```python
from build123d import *

# Parameters (mm, degrees)
BOSS_EXTRUDE1_DEPTH = 50
FILLET1_R           = 3
SKETCH3_R           = 2.5
CUT_EXTRUDE1_DEPTH  = 3
SKETCH4_R           = 1.5
CUT_EXTRUDE2_DEPTH  = 52.816130281
SKETCH5_R           = 1.5
CUT_EXTRUDE3_DEPTH  = 52.816130281
FILLET5_R           = 3
FILLET6_R           = 3
FILLET7_R           = 1


with BuildPart() as part:
    # Sketch1 → Boss-Extrude1 (new body)
    with BuildSketch(Plane.XY):
        Polygon((-4.736842105, 0), (-4.736842105, 6), (13.263157895, 6), (13.263157895, 0.55), (7.263157895, 0.55), (7.263157895, 0), align=None)
    extrude(amount=BOSS_EXTRUDE1_DEPTH)

    # Fillet1
    fillet1_edges = [part.edges().sort_by_distance(p)[0] for p in [
        (7.263157895, 0.275, 50),
    ]]
    fillet(fillet1_edges, radius=FILLET1_R)

    # Sketch3 → Cut-Extrude1 (cut)
    with BuildSketch(Plane(origin=(0, 6, 0), x_dir=(1, 0, 0), z_dir=(0, 1, 0))):
        with Locations(Location((0.263157895, -10, 0), (0, 0, 180))):
            Circle(SKETCH3_R)
        with Locations(Location((0.263157895, -40, 0), (0, 0, 180))):
            Circle(SKETCH3_R)
    extrude(amount=-CUT_EXTRUDE1_DEPTH, mode=Mode.SUBTRACT)

    # Sketch4 → Cut-Extrude2 (cut, through all)
    with BuildSketch(Plane(origin=(0, 3, 0), x_dir=(1, 0, 0), z_dir=(0, 1, 0))):
        with Locations(Location((0.263157895, -40, 0), (0, 0, 180))):
            Circle(SKETCH4_R)
    extrude(amount=-CUT_EXTRUDE2_DEPTH, mode=Mode.SUBTRACT)

    # Sketch5 → Cut-Extrude3 (cut, through all)
    with BuildSketch(Plane(origin=(0, 3, 0), x_dir=(1, 0, 0), z_dir=(0, 1, 0))):
        with Locations(Location((0.263157895, -10, 0), (0, 0, 180))):
            Circle(SKETCH5_R)
    extrude(amount=-CUT_EXTRUDE3_DEPTH, mode=Mode.SUBTRACT)

    # Fillet5
    fillet5_edges = [part.edges().sort_by_distance(p)[0] for p in [
        (7.263157895, 0.275, 0),
    ]]
    fillet(fillet5_edges, radius=FILLET5_R)

    # Fillet6
    fillet6_edges = [part.edges().sort_by_distance(p)[0] for p in [
        (-4.736842105, 3, 50),
        (-4.736842105, 3, 0),
    ]]
    fillet(fillet6_edges, radius=FILLET6_R)

    # Fillet7
    fillet7_edges = [part.edges().sort_by_distance(p)[0] for p in [
        (13.263157895, 6, 25),
        (5.763157895, 6, 50),
        (-4.736842105, 6, 25),
        (-3.858162449, 6, 49.121320344),
        (-3.858162449, 6, 0.878679656),
        (5.763157895, 6, 0),
    ]]
    fillet(fillet7_edges, radius=FILLET7_R)


solid = part.part
```
Part model, mm, in its own coordinate system. A direction names the side the tool comes from. Round coordinates to 2 decimals unless told otherwise and drop trailing zeros. Order: outer loops, then holes, each group sorted by start corner. A loop starts at its lowest first (then second) coordinate and runs counter-clockwise, first axis right, second up. Notation, with made-up numbers: M -5,64 L 10,64 A30 ccw 10,86 Z; hole C 73,39 d10. An arc over 180 degrees is marked long. Answer in a Markdown table with one row per item. Add a question column.
Q1. 3-axis set-ups, long thin cutter, end or side, ignore diameter. For faces 4 (the face through (0, 3, 8)), 5 (the face through (6.408, 0.271, 0.902)), 6 (the face through (6.408, 0.271, 49.098)): which of +Z, -Z, +X, -X, +Y, -Y reach the whole face in a straight line?
Q2. Cut at C-C on x = 11.25. Give the cut face in (y, z), and give its area (3 significant figures).
Q3. Mould opens along X. For faces 1 (the face through (13.263, 3, 25)), 2 (the face through (0.588, 1.521, 8.536)), 3 (the face through (5.658, 5.699, 0.285)) say: +X half, -X half, draft (parallel to the pull), parting line (faces both ways), or undercut.
Q4. Cut at B-B on y = 3.55. Give the cut face in (x, z), and give its area (3 significant figures).
Q5. Cut at A-A on z = 10. Give the cut face in (x, y), and give its area (3 significant figures).
Q6. Pin check, flat tips, straight feed: pin 1 (4 mm diameter, centred on x = 0.26, z = 10, fed in from +Y); pin 2 (4.5 mm diameter, centred on x = 11, z = 19.5, fed in from -Y); pin 3 (1.8 mm diameter, centred on x = 0.26, z = 40, fed in from +Y). Stop position of each tip, or through.
Q7. Wall check: L1, parallel to Z at x = -0.25, y = 1.45; L2, parallel to Z at x = 0, y = 5.1; L3, parallel to Y at x = 12, z = 20. Give the ranges that are in metal, low to high. Write a range as from..to.
Q8. Cut at D-D on z = 31.5. Give the cut face in (x, y).
Established:
| question | item | result |
|---|---|---|
| 1 | face 4 | +Y |
| 1 | face 5 | -Z, +X, -Y |
| 1 | face 6 | +Z, +X, -Y |
| 2 | outline | M 0.55,0 L 5,0 A1 ccw 6,1 L 6,49 A1 ccw 5,50 L 0.55,50 Z |
| 2 | area | 272 mm2 |
| 3 | face 1 | +X half |
| 3 | face 2 | undercut |
| 3 | face 3 | draft |
| 4 | outline | M -4.74,3 A3 ccw -1.74,0 L 13.26,0 L 13.26,50 L -1.74,50 A3 ccw -4.74,47 Z; hole C 0.26,10 d5; hole C 0.26,40 d5 |
| 4 | area | 857 mm2 |
| 5 | outline | M -4.74,0 L -1.24,0 L -1.24,3 L -2.24,3 L -2.24,6 L -3.74,6 A1 ccw -4.74,5 Z; M 1.76,0 L 7.26,0 L 7.26,0.55 L 13.26,0.55 L 13.26,5 A1 ccw 12.26,6 L 2.76,6 L 2.76,3 L 1.76,3 Z |
| 5 | area | 80.3 mm2 |
| 6 | pin 1 | stops at y = 3 |
| 6 | pin 2 | stops at y = 0.55 |
| 6 | pin 3 | passes through |
| 7 | L1 | z = 0..8.59, 11.41..38.59, 41.41..50 |
| 7 | L2 | z = 0.01..7.51, 12.49..37.51, 42.49..49.99 |
| 7 | L3 | y = 0.55..6 |
| 8 | outline | M -4.74,0 L 7.26,0 L 7.26,0.55 L 13.26,0.55 L 13.26,5 A1 ccw 12.26,6 L -3.74,6 A1 ccw -4.74,5 Z |
